Can you work these out from the drawing? Everything is in mm from the part's minimum corner. Coordinates: 2 decimals unless noted, no trailing zeros. Loops run counter-clockwise (first coordinate to the right, second up) from the corner with the lowest first, then second, coordinate; pieces in that order, holes last.
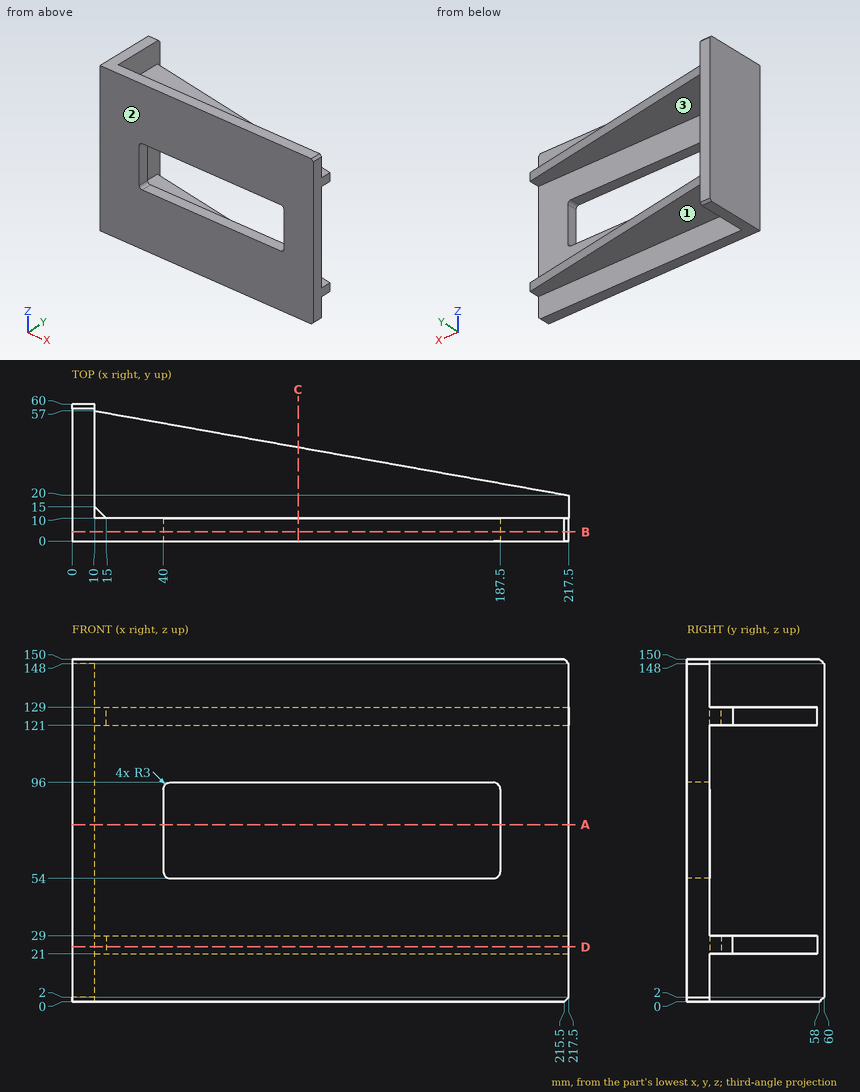
(1) Imagine slicing it at A-A, the plane z = 77.5. Write out the boundary of the cut face in (x, y).
Answers:
outline: (0, 0) - (40, 0) - (40, 10) - (10, 10) - (10, 60) - (0, 60) - close; (187.5, 0) - (217.5, 0) - (217.5, 10) - (187.5, 10) - close
(2) Imagine slicing it at B-B, the plane y = 4. Write out the boundary of the cut face in (x, z).
Answers:
outline: (0, 0) - (215.5, 0) - (217.5, 2) - (217.5, 148) - (215.5, 150) - (0, 150) - close; hole (40, 57) arc R3 ccw to (43, 54) - (184.5, 54) arc R3 ccw to (187.5, 57) - (187.5, 93) arc R3 ccw to (184.5, 96) - (43, 96) arc R3 ccw to (40, 93) - close
(3) For pin 1 (23.5 mm diameter, centred on x = 63.5, y = 43, fed in from -Z); pin 2 (1 mm diameter, centred on y = 44.5, z = 19, fed in from +X); pin 3 (2 mm diameter, centred on x = 96.5, z = 54, fed in from +Y), each with a flat end and sliding along its axis, tell me the tip position at first contact or that it passes through.
Answers:
pin 1: stops at z = 21
pin 2: stops at x = 10
pin 3: stops at y = 10
(4) I need wall thicknesses on probe 1 along Z at (x, y) = (47.5, 25); probe 2 along Z at (x, y) = (75, 8.5); probe 3 along Y at (x, z) = (46.5, 114.5). Which ranges of each line are inside material? Lowest first, please.
Answers:
probe 1: z = 21 to 29, 121 to 129
probe 2: z = 0 to 54, 96 to 150
probe 3: y = 0 to 10
(5) We'd pull the mould along Z, two halves only. Please class the marked faces 1, 2 and 3: +Z half, -Z half, draft (parallel to the pull), parting line (faces both ways), or undercut.
Answers:
face 1: -Z half
face 2: draft
face 3: undercut
(6) Imagine slicing it at C-C, the plane x = 99. Write out the boundary of the cut face in (y, z).
Answers:
outline: (0, 0) - (10, 0) - (10, 21) - (41.13, 21) - (41.13, 29) - (10, 29) - (10, 54) - (0, 54) - close; (0, 96) - (10, 96) - (10, 121) - (41.13, 121) - (41.13, 129) - (10, 129) - (10, 150) - (0, 150) - close
(7) Imagine slicing it at D-D, the plane z = 24. Write out the boundary of the cut face in (x, y), and give its area (3 significant figures).
Answers:
outline: (0, 0) - (217.5, 0) - (217.5, 20) - (10, 57) - (10, 60) - (0, 60) - close; hole (10, 10) - (15, 10) - (10, 15) - close
area: 8,580 mm2
